from build123d import *

# Parameters (mm, degrees)
EXTRUDE_1_DEPTH = 6


with BuildPart() as part:
    # 草图1 → 凸台-拉伸1 (new body)
    with BuildSketch(Plane(origin=(8, 0, 0), x_dir=(0, 0, -1), z_dir=(1, 0, 0))):
        Polygon((-8.660254038, 0), (-4.330127019, -7.5), (4.330127019, -7.5), (8.660254038, 0), (4.330127019, 7.5), (-4.330127019, 7.5), align=None)
    extrude(amount=-EXTRUDE_1_DEPTH)

    # 草图2 → 旋转1 (revolve)
    with BuildSketch(Plane.XY, mode=Mode.PRIVATE) as revolve_1_sk:
        Polygon((-15, 5), (-15, 0), (2, 0), (2, 4.157220044), (0, 4.157220044), (0, 5), align=None)
    revolve(revolve_1_sk.sketch.rotate(Axis((-15, 0, 0), (1, 0, 0)), 270), axis=Axis((-15, 0, 0), (1, 0, 0)))

    # 草图3 → 旋转2 (revolve)
    with BuildSketch(Plane.XY, mode=Mode.PRIVATE) as revolve_2_sk:
        Polygon((8, 4.157220044), (8, 0), (20, 0), (20, 5), (10, 5), (10, 4.157220044), align=None)
    revolve(revolve_2_sk.sketch.rotate(Axis((8, 0, 0), (1, 0, 0)), 270), axis=Axis((8, 0, 0), (1, 0, 0)))


solid = part.part
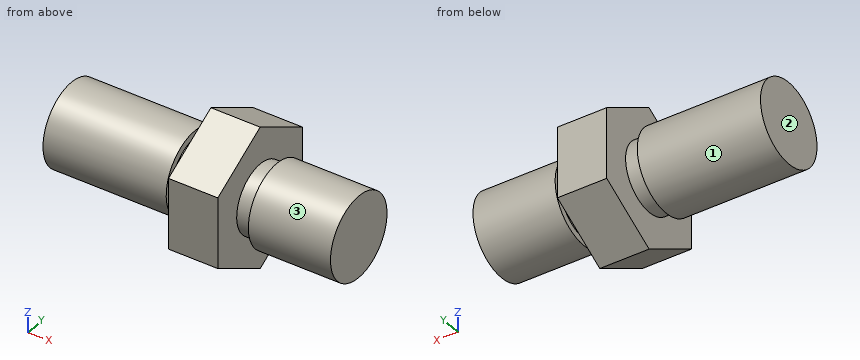
Source: CAD feature listing. Evaluate the final solid. Frame: model axes, mm. Face numbers are marked on the shaded views. A direction names the side the tool comes from. Round coordinates to 2 decimals unless told otherwise and drop trailing zeros. Loops run counter-clockwise (first coordinate to the right, second up) from the corner with the lowest first, then second, coordinate; pieces in that order, holes last.
Q1. Section C-C, the plane y = 2.75. Return loops of the section in (x, z).
Q2. Section D-D, the plane x = 10.5. Return loops of the section in (y, z).
Q3. Access query for the marked faces 1, 2 and 3. Directions: +Z, -Z, +X, -X, +Y, -Y. A direction counts if a zero-diameter tool reaches every point of the face in a straight line with its end or side. Return the directions, or none.
Q4. First-contact query: P1, Ø4, axis at y = 5.5, z = 6, coming from the +X side; P2, Ø1, axis at x = 10.5, z = 4, coming from the +Y side; P3, Ø10, axis at x = -5, z = -1.5, coming from the -Y side. Flat tips, straight axial feed; report the tip coordinate or a pass-through.
Q5. Section A-A, the plane z = 0. Return loops of the section in (x, y).
Q6. Ray query, line 1 (X direction, y = 4.5, z = 1); line 2 (X direction, y = 6.5, z = 4.5); line 3 (Y direction, x = 17, z = -2.25). Return the intervals inside material, ascending.
Q7. Section B-B, the plane x = 4. Return loops of the section in (y, z).
Solutions:
1. outline: (-15, -4.18) - (0, -4.18) - (0, -3.12) - (2, -3.12) - (2, -7.07) - (8, -7.07) - (8, -3.12) - (10, -3.12) - (10, -4.18) - (20, -4.18) - (20, 4.18) - (10, 4.18) - (10, 3.12) - (8, 3.12) - (8, 7.07) - (2, 7.07) - (2, 3.12) - (0, 3.12) - (0, 4.18) - (-15, 4.18) - close
2. outline: circle Ø10 at (0, 0)
3. face 1: -X
3. face 2: +Z, -Z, -X, +Y, -Y
3. face 3: +X
4. P1: stops at x = 8
4. P2: stops at y = 3.57
4. P3: stops at y = -5
5. outline: (-15, -5) - (0, -5) - (0, -4.16) - (2, -4.16) - (2, -7.5) - (8, -7.5) - (8, -4.16) - (10, -4.16) - (10, -5) - (20, -5) - (20, 5) - (10, 5) - (10, 4.16) - (8, 4.16) - (8, 7.5) - (2, 7.5) - (2, 4.16) - (0, 4.16) - (0, 5) - (-15, 5) - close
6. line 1: x = -15 to 0, 2 to 8, 10 to 20
6. line 2: x = 2 to 8
6. line 3: y = -4.47 to 4.47
7. outline: (-7.5, -4.33) - (0, -8.66) - (7.5, -4.33) - (7.5, 4.33) - (0, 8.66) - (-7.5, 4.33) - close
